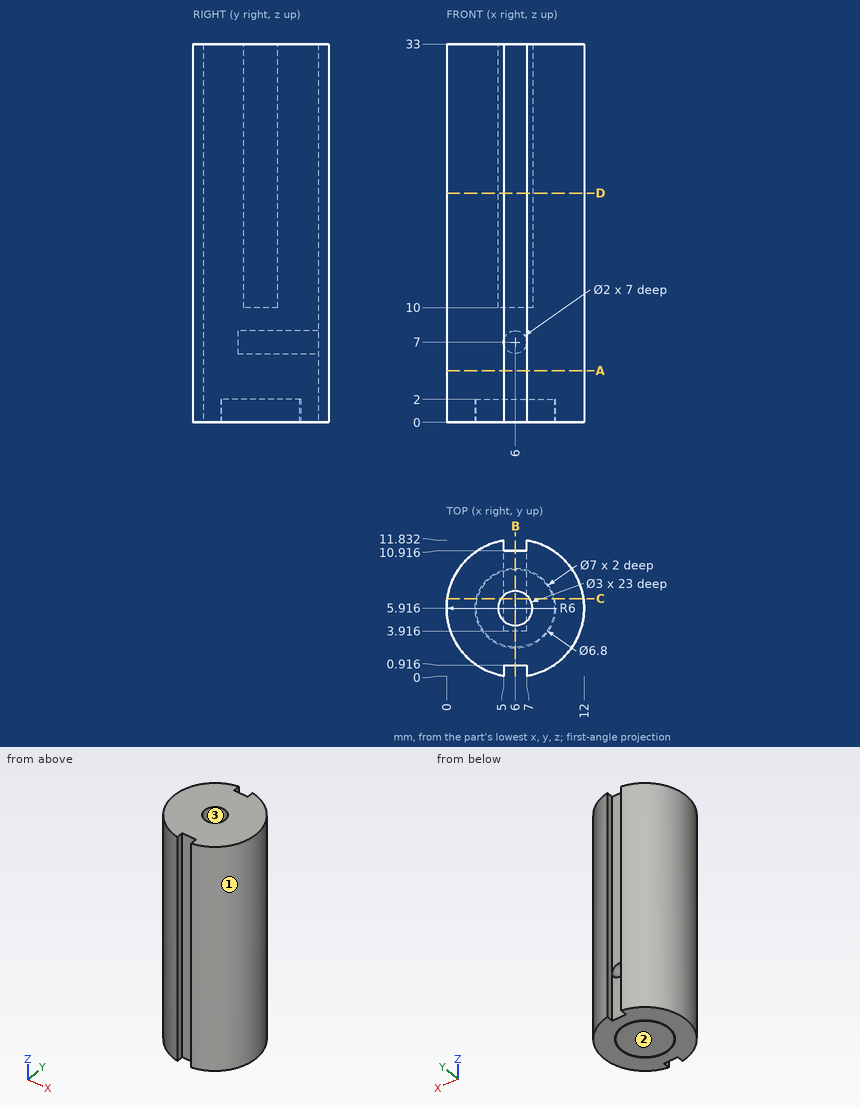
Answer from the drawing. Dimensions are ordinates in mm from the lowest x, y and z of the part. Give positions to 0.01 mm unless a question says otherwise; leave off trailing zeros. Order: outer loops, then holes, each group sorted by start corner. A loop starts at its lowest first (then second) coordinate and runs counter-clockwise, first axis right, second up. Notation, with made-up numbers: (-17.5, 38) - (28.5, 38) arc R11 cw to (28.5, 45) - close; hole circle Ø3 at (68, 53.5). An arc over 180 degrees is marked (long way). One line per item, written item: value. Start each with the question number.
1) A cutting plane is placed at C-C on y = 6.75. Give the vertices of the cut face in (x, z).
2) A cutting plane is placed at D-D on z = 20. Give the vertices of the cut face in (x, y), then the cut area to 3 significant figures.
3) The mould has two halves that part along Y. Classify the marked faces 1, 2 and 3: released by +Y, released by -Y, zero draft, split by the parting line, or undercut.
4) A cutting plane is placed at B-B on x = 6. Give the vertices of the cut face in (y, z), then the cut area to 3 significant figures.
5) Find the intervals of material crossed by L1, parallel to Y at x = 6, z = 23.75; L2, parallel to X at y = 6.75, z = 17; L3, parallel to Y at x = 5.25, z = 10.5 (1 decimal), in increasing order.
6) A cutting plane is placed at A-A on z = 4.5. Give the vertices of the cut face in (x, y), then the cut area to 3 significant figures.
7) Given pin 1 Ø1.2 at (x, z) = (6, 7) entering from +Y; pin 2 Ø1 at (y, z) = (11.5, 12.5) entering from -X; pin 3 Ø4 at (x, y) = (7, 8.5) entering from -Z; pin 4 Ø6 at (y, z) = (2.5, 17) entering from -X, each flat-ended and moving along its own axis, determine where each tip first touches the part or whether it passes through.
Answer sheet:
1. outline: (0.06, 0) - (2.6, 0) - (2.6, 2) - (2.7, 2) - (2.7, 0) - (9.3, 0) - (9.3, 2) - (9.4, 2) - (9.4, 0) - (11.94, 0) - (11.94, 33) - (7.25, 33) - (7.25, 10) - (4.75, 10) - (4.75, 33) - (0.06, 33) - close; hole circle Ø2 at (6, 7)
2. outline: (5, 0) - (5, 0.92) - (7, 0.92) - (7, 0) arc R6 ccw to (7, 11.83) - (7, 10.92) - (5, 10.92) - (5, 11.83) arc R6 ccw to start; hole circle Ø3 at (6, 5.92)
2. area: 102 mm2
3. face 1: split by the parting line
3. face 2: zero draft
3. face 3: undercut
4. outline: (0.92, 0) - (2.42, 0) - (2.42, 2) - (2.52, 2) - (2.52, 0) - (9.32, 0) - (9.32, 2) - (9.42, 2) - (9.42, 0) - (10.92, 0) - (10.92, 6) - (3.92, 6) - (3.92, 8) - (10.92, 8) - (10.92, 33) - (7.42, 33) - (7.42, 10) - (4.42, 10) - (4.42, 33) - (0.92, 33) - close
4. area: 247 mm2
5. L1: y = 0.92 to 4.42, 7.42 to 10.92
5. L2: x = 0.06 to 4.75, 7.25 to 11.94
5. L3: y = 0.9 to 4.6, 7.2 to 10.9
6. outline: (5, 0) - (5, 0.92) - (7, 0.92) - (7, 0) arc R6 ccw to (7, 11.83) - (7, 10.92) - (5, 10.92) - (5, 11.83) arc R6 ccw to start
6. area: 109 mm2
7. pin 1: stops at y = 3.92
7. pin 2: stops at x = 2.81
7. pin 3: stops at z = 0
7. pin 4: stops at x = 0.01
